Build history of the part. All positions in model axes, mm. A direction names the side the tool comes from. Give positions to 0.01 mm unless a question says otherwise; leave off trailing zeros. Loops run counter-clockwise (first coordinate to the right, second up) from the corner with the lowest first, then second, coordinate; pieces in that order, holes last. Notation, with made-up numbers: (73.5, 86.5) - (84.5, 86.5) arc R14 ccw to (84.5, 98.5) - close; hole circle Ø2 at (64.5, 89). An arc over 180 degrees is marked (long way). Return JSON: item names as keys, results as strings. Group by question number.
1) Slice it at C-C (z = 7). List the corners of the cut face in (x, y).
2) Drop flat-ended pins along their axis: pin 1 (4 mm diameter, centred on x = -11, y = 52.5, fed in from +Z); pin 2 (1 mm diameter, centred on x = -35, z = 8.5, fed in from -Y); pin 3 (10 mm diameter, centred on x = -23, z = 16, fed in from -Y). Give the stop position or say it passes through.
3) Slice it at D-D (x = 0). List the corners of the cut face in (y, z).
4) Slice it at B-B (x = -10). List the corners of the cut face in (y, z), and give its area (3 significant figures).
5) 3-axis set-ups, long thin cutter, end or side, ignore diameter. For faces 1 (the face through (-1, 50, 18)), 2 (the face through (1.63, 47.7, 4.44)), 3 (the face through (-29.97, -18.68, 4.51)), 4 (the face through (-1, 67.02, 10)), 5 (the face through (32.08, 51.03, 13.56)): which of +Z, -Z, +X, -X, +Y, -Y reach the whole face in a straight line?
6) Slice it at A-A (y = -20). List the corners of the cut face in (x, z), and give its area (3 significant figures).
7) Drill centre lines: probe 1 along Y at (x, z) = (0, 2.1); probe 2 along Y at (x, z) = (0, 6); probe 3 along Y at (x, z) = (-11.5, 14.25). Where is each one in solid material? Low to high. Write a range as from..to.
8) Mould opens along X. For faces 6 (the face through (-1, 17, 20)), 7 (the face through (-36.445, -50.979, 10.14)), 8 (the face through (-28.37, 47.7, 4.44)) say: released by +X, released by -X, zero draft, split by the parting line, or undercut.
```python
from build123d import *

# Parameters (mm, degrees)
SKETCH1_W                                            = 90
SKETCH1_H                                            = 120
BOSS_EXTRUDE1_DEPTH                                  = 20
SKETCH2_R                                            = 34
CUT_EXTRUDE1_DEPTH                                   = 15
SKETCH3_R                                            = 30
CUT_EXTRUDE2_DEPTH                                   = 1
SKETCH4_R                                            = 14
CUT_EXTRUDE3_DEPTH                                   = 10
MOVE_FACE1_BY                                        = 2.02
FILLET1_R                                            = 30
MOVE_FACE2_BY                                        = 5
CBORE_FOR_M8_HEXAGON_SOCKET_HEAD_CAP_SCR_D           = 9
CBORE_FOR_M8_HEXAGON_SOCKET_HEAD_CAP_SCR_DEPTH       = 80.25
CBORE_FOR_M8_HEXAGON_SOCKET_HEAD_CAP_SCR_CBORE_D     = 15
CBORE_FOR_M8_HEXAGON_SOCKET_HEAD_CAP_SCR_CBORE_DEPTH = 9
CBORE_FOR_M8_HEXAGON_SOCKET_HEAD_CAP_SCR_TIP         = 2.703872786
SKETCH7_W                                            = 90
SKETCH7_H                                            = 14
CUT_EXTRUDE4_DEPTH                                   = 2


with BuildPart() as part:
    # Sketch1 → Boss-Extrude1 (new body)
    with BuildSketch(Plane.XY):
        Rectangle(SKETCH1_W, SKETCH1_H)
    extrude(amount=BOSS_EXTRUDE1_DEPTH)

    # Sketch2 → Cut-Extrude1 (cut)
    with BuildSketch(Plane.XY.offset(20)):
        with Locations((0, -20)):
            Circle(SKETCH2_R)
    extrude(amount=-CUT_EXTRUDE1_DEPTH, mode=Mode.SUBTRACT)

    # Sketch3 → Cut-Extrude2 (cut)
    with BuildSketch(Plane.XY.offset(5)):
        with Locations((0, -20)):
            Circle(SKETCH3_R)
    extrude(amount=-CUT_EXTRUDE2_DEPTH, mode=Mode.SUBTRACT)

    # Sketch4 → Cut-Extrude3 (cut)
    with BuildSketch(Plane.XY.offset(4)):
        with Locations((0, -20)):
            Circle(SKETCH4_R)
    extrude(amount=-CUT_EXTRUDE3_DEPTH, mode=Mode.SUBTRACT)

    # Move Face1: a face moved outward by 2.02
    extrude(part.faces().sort_by_distance((0, 60, 10))[0], amount=MOVE_FACE1_BY, dir=(0, 1, 0))

    # Fillet1
    fillet1_edges = [part.edges().sort_by_distance(p)[0] for p in [
        (45, -60, 10),
        (-45, -60, 10),
    ]]
    fillet(fillet1_edges, radius=FILLET1_R)

    # Move Face2: a face moved outward by 5.0
    extrude(part.faces().sort_by_distance((0, 62.02, 10))[0], amount=MOVE_FACE2_BY, dir=(0, 1, 0))

    # CBORE for M8 Hexagon socket head cap screws1
    with Locations(Plane(origin=(0, 0, 0), x_dir=(-1, 0, 0), z_dir=(0, 0, -1))):
        with Locations((30, 55.02), (-30, 55.02), (0, 55.02)):
            CounterBoreHole(CBORE_FOR_M8_HEXAGON_SOCKET_HEAD_CAP_SCR_D / 2, CBORE_FOR_M8_HEXAGON_SOCKET_HEAD_CAP_SCR_CBORE_D / 2, CBORE_FOR_M8_HEXAGON_SOCKET_HEAD_CAP_SCR_CBORE_DEPTH, depth=CBORE_FOR_M8_HEXAGON_SOCKET_HEAD_CAP_SCR_DEPTH)
            with Locations((0, 0, -(CBORE_FOR_M8_HEXAGON_SOCKET_HEAD_CAP_SCR_DEPTH + CBORE_FOR_M8_HEXAGON_SOCKET_HEAD_CAP_SCR_TIP / 2))):  # 118° drill point
                Cone(0, CBORE_FOR_M8_HEXAGON_SOCKET_HEAD_CAP_SCR_D / 2, CBORE_FOR_M8_HEXAGON_SOCKET_HEAD_CAP_SCR_TIP, mode=Mode.SUBTRACT)

    # Sketch7 → Cut-Extrude4 (cut)
    with BuildSketch(Plane.XY.offset(20)):
        with Locations((0, 55.02)):
            Rectangle(SKETCH7_W, SKETCH7_H)
    extrude(amount=-CUT_EXTRUDE4_DEPTH, mode=Mode.SUBTRACT)


solid = part.part
```
Results:
{
 "1": {"outline": "(-45, -30) arc R30 ccw to (-15, -60) - (15, -60) arc R30 ccw to (45, -30) - (45, 67.02) - (-45, 67.02) - close; hole circle Ø15 at (-30, 55.02); hole circle Ø68 at (0, -20); hole circle Ø15 at (0, 55.02); hole circle Ø15 at (30, 55.02)"},
 "2": {"pin 1": "z = 18", "pin 2": "y = -52.8", "pin 3": "y = -59.85"},
 "3": {"outline": "(-60, 0) - (-34, 0) - (-34, 4) - (-50, 4) - (-50, 5) - (-54, 5) - (-54, 20) - (-60, 20) - close; (-6, 0) - (47.52, 0) - (47.52, 9) - (50.52, 9) - (50.52, 18) - (48.02, 18) - (48.02, 20) - (14, 20) - (14, 5) - (10, 5) - (10, 4) - (-6, 4) - close; (59.52, 9) - (62.52, 9) - (62.52, 0) - (67.02, 0) - (67.02, 20) - (62.02, 20) - (62.02, 18) - (59.52, 18) - close"},
 "4": {"outline": "(-60, 0) - (-29.8, 0) - (-29.8, 4) - (-48.28, 4) - (-48.28, 5) - (-52.5, 5) - (-52.5, 20) - (-60, 20) - close; (-10.2, 0) - (67.02, 0) - (67.02, 20) - (62.02, 20) - (62.02, 18) - (48.02, 18) - (48.02, 20) - (12.5, 20) - (12.5, 5) - (8.28, 5) - (8.28, 4) - (-10.2, 4) - close", "area": "1,400 mm2"},
 "5": {"face 1": "+Z, +X, -X", "face 2": "-Z", "face 3": "+Z", "face 4": "+Z, -Z, +X, -X, +Y", "face 5": "+Z, -Z"},
 "6": {"outline": "(-45, 0) - (-14, 0) - (-14, 4) - (-30, 4) - (-30, 5) - (-34, 5) - (-34, 20) - (-45, 20) - close; (14, 0) - (45, 0) - (45, 20) - (34, 20) - (34, 5) - (30, 5) - (30, 4) - (14, 4) - close", "area": "608 mm2"},
 "7": {"probe 1": "-60..-34, -6..47.52, 62.52..67.02", "probe 2": "-60..-54, 14..47.52, 62.52..67.02", "probe 3": "-60..-52, 12..67.02"},
 "8": {"face 6": "zero draft", "face 7": "released by -X", "face 8": "undercut"}
}
